Print and shaded views of the part. All mm, measured from the part's lowest x, y and z. Round coordinates to 2 decimals unless told otherwise and drop trailing zeros. Write each loop counter-clockwise with the first axis right and the second up, starting at its lowest first coordinate (ties: lowest second). Pieces come first, ordered by that corner, then holes. Notation, with made-up numbers: (28.5, 45) - (72.5, 45) arc R21 cw to (72.5, 84) - close; hole circle Ø2 at (-33.75, 29.25). An arc over 180 degrees is marked (long way). One line per item, written item: value.
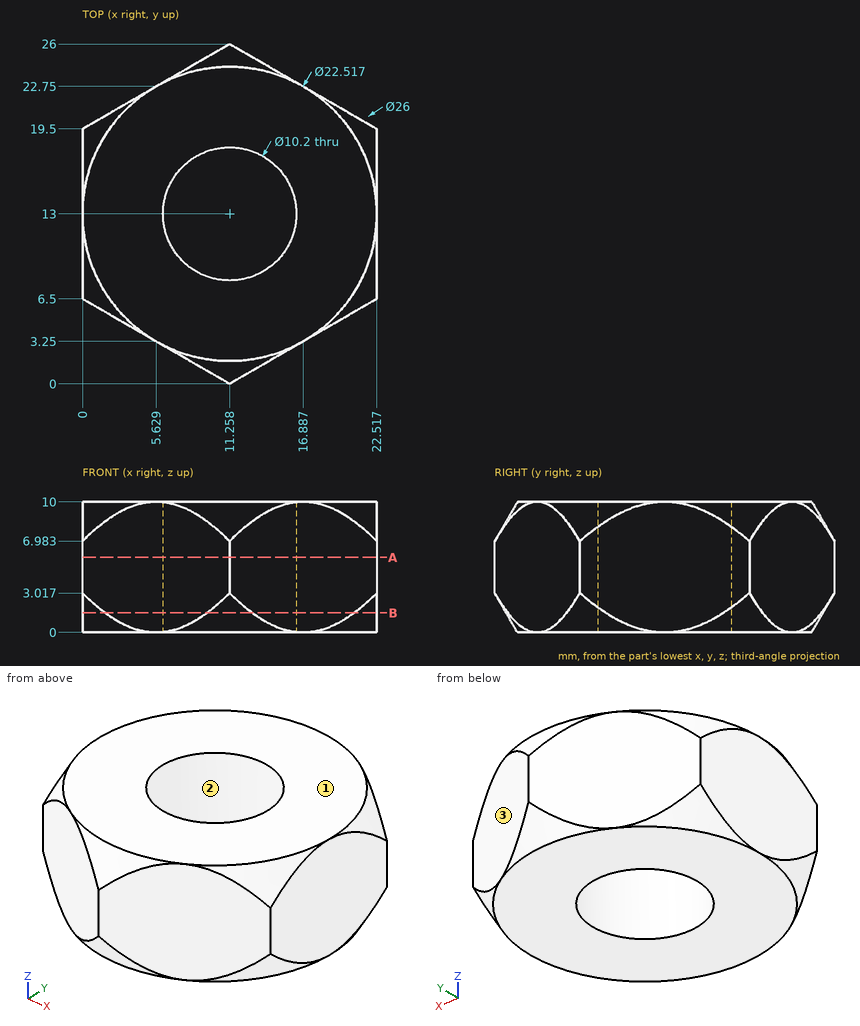
1. Band-saw the part on B-B on z = 1.5. Write the cut outline in (x, y) (1 decimal), plus the area to 3 significant figures.
Report:
outline: (0, 8.5) arc R12.1 ccw to (1.7, 5.5) - (9.5, 1) arc R12.1 ccw to (13, 1) - (20.8, 5.5) arc R12.1 ccw to (22.5, 8.5) - (22.5, 17.5) arc R12.1 ccw to (20.8, 20.5) - (13, 25) arc R12.1 ccw to (9.5, 25) - (1.7, 20.5) arc R12.1 ccw to (0, 17.5) - close; hole circle Ø10.2 at (11.3, 13)
area: 349 mm²
2. Wall check: probe 1 along X at (y, z) = (13.5, 1); probe 2 along X at (y, z) = (11.5, 4.25) (1 decimal); probe 3 along Y at (x, z) = (8, 6) (1 decimal). Give the ranges that are in metal, low to high. Write a range as [from, to].
Report:
probe 1: [0, 6.18], [16.33, 22.52]
probe 2: [0, 6.4], [16.1, 22.5]
probe 3: [1.9, 9.1], [16.9, 24.1]
3. Mould opens along Y. For the marked faces 1, 2 and 3 say: released by +Y, released by -Y, zero draft, split by the parting line, or undercut.
Report:
face 1: zero draft
face 2: undercut
face 3: released by +Y
4. Drop flat-ended pins along their axis: pin 1 (2 mm diameter, centred on x = 11, z = 1.5, fed in from +Y); pin 2 (4 mm diameter, centred on x = 18.5, z = 4, fed in from +Y) (1 decimal); pin 3 (4 mm diameter, centred on x = 7, z = 6.5, fed in from +Y) (1 decimal). Give the stop position or say it passes through.
Report:
pin 1: y = 25.7
pin 2: y = 23
pin 3: y = 24.7
5. Band-saw the part on A-A on z = 5.75. Write the cut outline in (x, y), plus the area to 3 significant figures.
Report:
outline: (0, 6.5) - (11.26, 0) - (22.52, 6.5) - (22.52, 19.5) - (11.26, 26) - (0, 19.5) - close; hole circle Ø10.2 at (11.26, 13)
area: 357 mm²
